Could you check a few things on this model? Use its own coordinates, in mm. Give positions to 0.01 mm unless a question says otherwise; leave off trailing zeros. Order: outer loops, then holes, each group sorted by start corner. A loop starts at its lowest first (then second) coordinate and runs counter-clockwise, first axis right, second up. Notation, with made-up numbers: M 30.25,64 L 50.25,64 A22 cw 50.25,92 Z; hole C 42,31 d3. An arc over 180 degrees is marked long. Use a Markdown table: item, result. Add a question column.
Item 1: Suppose I cut it at A-A on z = 732.5. Write out the boundary of the cut face in (x, y).
Item 2: If I drill on L1, parallel to Z at x = -5.5, y = 10.5; L2, parallel to Z at x = 14, y = 13; L3, parallel to Y at x = 2, z = 206.5, over which ranges is the centre line in solid material (lowest first)? Write a range as from..to.
Item 3: I'm going to push flat-ended pins straight in: pin 1 Ø3 at (x, z) = (-10.5, 504) entering from +Y; pin 2 Ø8 at (y, z) = (0.5, 751) entering from -X; pin 3 Ø4 at (x, z) = (-17, 277) entering from -Y. Where does each tip first touch, or does it pass through?
Item 4: Suppose I cut it at B-B on y = 0. Write out the boundary of the cut face in (x, z).
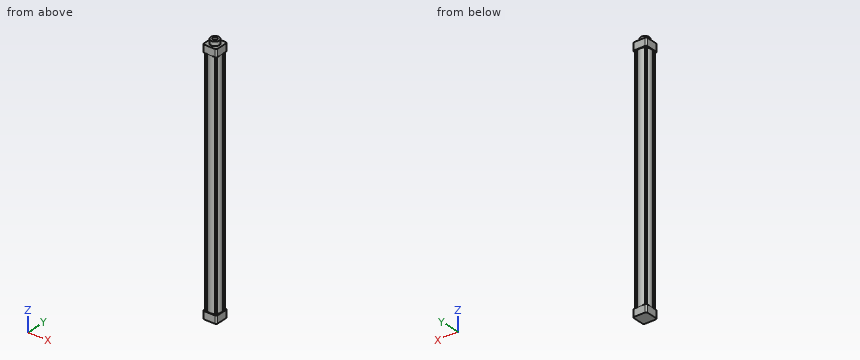
from build123d import *

# Parameters (mm, degrees)
SKETCH1_W           = 50
SKETCH1_H           = 50
BOSS_EXTRUDE1_DEPTH = 27.5
SKETCH2_R           = 23
SKETCH2_R_2         = 20
BOSS_EXTRUDE2_DEPTH = 860
SKETCH3_W           = 50
SKETCH3_H           = 50
BOSS_EXTRUDE3_DEPTH = 27.5
SKETCH4_R           = 16
BOSS_EXTRUDE4_DEPTH = 15
SKETCH5_R           = 8
CUT_EXTRUDE1_DEPTH  = 100
SKETCH6_R           = 3
BOSS_EXTRUDE5_DEPTH = 915
FILLET1_R           = 5


with BuildPart() as part:
    # Sketch1 → Boss-Extrude1 (new body)
    with BuildSketch(Plane.XY):
        Rectangle(SKETCH1_W, SKETCH1_H)
    extrude(amount=BOSS_EXTRUDE1_DEPTH)

    # Sketch2 → Boss-Extrude2 (add)
    with BuildSketch(Plane.XY.offset(27.5)):
        Circle(SKETCH2_R)
        Circle(SKETCH2_R_2, mode=Mode.SUBTRACT)
    extrude(amount=BOSS_EXTRUDE2_DEPTH)

    # Sketch3 → Boss-Extrude3 (add)
    with BuildSketch(Plane.XY.offset(887.5)):
        Rectangle(SKETCH3_W, SKETCH3_H)
    extrude(amount=BOSS_EXTRUDE3_DEPTH)

    # Sketch4 → Boss-Extrude4 (add)
    with BuildSketch(Plane.XY.offset(915)):
        Circle(SKETCH4_R)
    extrude(amount=BOSS_EXTRUDE4_DEPTH)

    # Sketch5 → Cut-Extrude1 (cut)
    with BuildSketch(Plane.XY.offset(930)):
        Circle(SKETCH5_R)
    extrude(amount=-CUT_EXTRUDE1_DEPTH, mode=Mode.SUBTRACT)

    # Sketch6 → Boss-Extrude5 (add)
    with BuildSketch(Plane.XY.offset(915)):
        with Locations((-18.5, 18.5)):
            Circle(SKETCH6_R)
        with Locations((18.5, 18.5)):
            Circle(SKETCH6_R)
        with Locations((18.5, -18.5)):
            Circle(SKETCH6_R)
        with Locations((-18.5, -18.5)):
            Circle(SKETCH6_R)
    extrude(amount=-BOSS_EXTRUDE5_DEPTH)

    # Fillet1
    fillet1_edges = [part.edges().sort_by_distance(p)[0] for p in [
        (25, -25, 901.25),
        (25, 25, 901.25),
        (-25, 25, 901.25),
        (-25, -25, 901.25),
        (25, -25, 13.75),
        (-25, -25, 13.75),
        (-25, 25, 13.75),
        (25, 25, 13.75),
    ]]
    fillet(fillet1_edges, radius=FILLET1_R)


solid = part.part
Findings below:
| question | item | result |
|---|---|---|
| 1 | outline | C 0,0 d46; C -18.5,-18.5 d6; C -18.5,18.5 d6; C 18.5,-18.5 d6; C 18.5,18.5 d6; hole C 0,0 d40 |
| 2 | L1 | z = 0..27.5, 887.5..930 |
| 2 | L2 | z = 0..27.5, 887.5..915 |
| 2 | L3 | y = -22.91..-19.9, 19.9..22.91 |
| 3 | pin 1 | stops at y = 21.17 |
| 3 | pin 2 | stops at x = -23 |
| 3 | pin 3 | stops at y = -21.5 |
| 4 | outline | M -25,0 L 25,0 L 25,27.5 L 23,27.5 L 23,887.5 L 25,887.5 L 25,915 L 16,915 L 16,930 L 8,930 L 8,887.5 L 20,887.5 L 20,27.5 L -20,27.5 L -20,887.5 L -8,887.5 L -8,930 L -16,930 L -16,915 L -25,915 L -25,887.5 L -23,887.5 L -23,27.5 L -25,27.5 Z |
